Could you check a few things on this model? Use its own coordinates, in mm. A direction names the side the tool comes from. Round coordinates to 2 decimals unless told otherwise and drop trailing zeros. Answer in a Markdown table with one row per item.
from build123d import *

# Parameters (mm, degrees)
CONECUT_DEPTH      = 68.537026869
CONECUT_DEPTH_BACK = 68.537026869


with BuildPart() as part:
    # Body: sweep along a path in 草图2
    with BuildLine(Plane.XY) as body_path:
        Line((63, 4), (0, 4))
        ThreePointArc((0, 4), (-1.740570538, 4.344328693), (-3.218934911, 5.325443787))
        ThreePointArc((-3.218934911, 5.325443787), (-16, 0), (-3.218934911, -5.325443787))
        ThreePointArc((-3.218934911, -5.325443787), (-1.740570538, -4.344328693), (0, -4))
        Line((0, -4), (67, -4))
    # 草图1 → Body (sweep)
    with BuildSketch(Plane(origin=(63, 0, 0), x_dir=(0, 0, -1), z_dir=(1, 0, 0))):
        with BuildLine():
            Line((-3.9999995, 0.002), (3.9999995, 0.002))
            ThreePointArc((3.9999995, 0.002), (0, 4), (-3.9999995, 0.002))
        make_face()
    sweep(path=body_path.line)

    # 草图3 → ConeCut (cut, two sides: drawn at the far end of the back side and taken through both)
    with BuildSketch(Plane.XY.offset(-CONECUT_DEPTH_BACK)):
        Polygon((63, 2.001), (60.139364077, 4.01), (67.01, 4.01), (67.01, -4.01), (64.139364077, -4.01), (67, -2.001), (64.133762416, 0), (60.133762416, 0), align=None)
    extrude(amount=CONECUT_DEPTH + CONECUT_DEPTH_BACK, mode=Mode.SUBTRACT)


solid = part.part
1) For faces 1 (the face through (61.913, 2.764, -0.048)), 2 (the face through (31, 4, 0)), 3 (the face through (34, -4, 0)), which set-ups out of +Z, -Z, +X, -X, +Y, -Y let a thin tool reach every point of the face, with its end or its side?
Findings:
| item | result |
|---|---|
| face 1 | +Z, -Z, +X, +Y |
| face 2 | +X, +Y |
| face 3 | +X, -Y |
2) For pin 1 (2 mm diameter, centred on x = 27.5, z = 3, fed in from +Y); pin 2 (4 mm diameter, centred on x = 24, z = -0.5, fed in from -Y), each with a flat end and sliding along its axis, tell me the tip position at first contact or that it passes through.
Findings:
| item | result |
|---|---|
| pin 1 | stops at y = 3.46 |
| pin 2 | stops at y = -4 |
3) Please list where these lines run through material, in increasing order: line 1 (Y direction, x = -8.5, z = 0); line 2 (Z direction, x = 35, y = 2); line 3 (Y direction, x = -8.5, z = -1.25).
Findings:
| item | result |
|---|---|
| line 1 | y = -7.5 to -3.5, 3.5 to 7.5 |
| line 2 | z = -3.46 to 3.46 |
| line 3 | y = -7.3 to -3.5, 3.5 to 7.3 |
